```python
from build123d import *

# Parameters (mm, degrees)
SKETCH_1_W                   = 23
SKETCH_1_H                   = 20
EXTRUDE_1_DEPTH              = 11
HOLE_WIZARD_M6_1_D           = 6.6
HOLE_WIZARD_M6_1_CBORE_D     = 11
HOLE_WIZARD_M6_1_CBORE_DEPTH = 6.4
CHAMFER_1_SIZE               = 2


with BuildPart() as part:
    # 草图1 → 凸台-拉伸1 (new, symmetric)
    with BuildSketch(Plane(origin=(0, 0, 0), x_dir=(1, 0, 0), z_dir=(0, 1, 0))):
        Rectangle(SKETCH_1_W, SKETCH_1_H)
    extrude(amount=EXTRUDE_1_DEPTH, both=True)

    # M6 六角凹头螺钉的柱形沉头孔1 (through all)
    with Locations(Plane(origin=(0, 11, 0), x_dir=(1, 0, 0), z_dir=(0, 1, 0))):
        with Locations((0, 0)):
            CounterBoreHole(HOLE_WIZARD_M6_1_D / 2, HOLE_WIZARD_M6_1_CBORE_D / 2, HOLE_WIZARD_M6_1_CBORE_DEPTH)

    # 倒角1
    chamfer_1_edges = [part.edges().sort_by_distance(p)[0] for p in [
        (-11.5, 0, -10),
        (11.5, 0, -10),
        (11.5, 0, 10),
        (-11.5, 0, 10),
    ]]
    chamfer(chamfer_1_edges, length=CHAMFER_1_SIZE)


solid = part.part
```
Build history of the part. All positions in model axes, mm. A direction names the side the tool comes from. Coordinates: 2 decimals unless noted, no trailing zeros. Write each loop counter-clockwise with the first axis right and the second up, starting at its lowest first coordinate (ties: lowest second). Pieces come first, ordered by that corner, then holes.
1. Drill centre lines: probe 1 along Z at (x, y) = (0, 7.5); probe 2 along X at (y, z) = (10, -0.25); probe 3 along Z at (x, y) = (0, -2.25). Where is each one in solid material? Low to high.
Answer block:
probe 1: z = -10 to -5.5, 5.5 to 10
probe 2: x = -11.5 to -5.49, 5.49 to 11.5
probe 3: z = -10 to -3.3, 3.3 to 10
2. 3-axis set-ups, long thin cutter, end or side, ignore diameter. For faces 4 (the cylindrical face through (-1.19, 7.84, 5.37)), 5 (the flat face through (-10.5, 0.2, -9)): which of +Z, -Z, +X, -X, +Y, -Y reach the whole face in a straight line?
Answer block:
face 4: +Y
face 5: -Z, -X, +Y, -Y
3. Pull direction Z, two halves, no side cores. Call faces 1 (the flat face through (0, 0, -10)), 2 (the flat face through (4, 4.6, 0)), 3 (the flat face through (0, 0, 10)): released by +Z, released by -Z, zero draft, split by the parting line, or undercut.
Answer block:
face 1: released by -Z
face 2: undercut
face 3: released by +Z
4. Band-saw the part on B-B, the plane y = -0.75. Give the cut face in (x, z), and give its area (3 significant figures).
Answer block:
outline: (-11.5, -8) - (-9.5, -10) - (9.5, -10) - (11.5, -8) - (11.5, 8) - (9.5, 10) - (-9.5, 10) - (-11.5, 8) - close; hole circle Ø6.6 at (0, 0)
area: 418 mm2
5. Band-saw the part on A-A, the plane z = 0. Give the cut face in (x, y).
Answer block:
outline: (-11.5, -11) - (-3.3, -11) - (-3.3, 4.6) - (-5.5, 4.6) - (-5.5, 11) - (-11.5, 11) - close; (3.3, -11) - (11.5, -11) - (11.5, 11) - (5.5, 11) - (5.5, 4.6) - (3.3, 4.6) - close
6. Band-saw the part on C-C, the plane x = 0. Give the cut face in (y, z), and give its area (3 significant figures).
Answer block:
outline: (-11, -10) - (11, -10) - (11, -5.5) - (4.6, -5.5) - (4.6, -3.3) - (-11, -3.3) - close; (-11, 3.3) - (4.6, 3.3) - (4.6, 5.5) - (11, 5.5) - (11, 10) - (-11, 10) - close
area: 267 mm2
7. Band-saw the part on D-D, the plane x = 10. Give the cut face in (y, z), and give its area (3 significant figures).
Answer block:
outline: (-11, -9.5) - (11, -9.5) - (11, 9.5) - (-11, 9.5) - close
area: 418 mm2
